```python
from build123d import *

# Parameters (mm, degrees)
BASEHEAD_DEPTH     = 3.5
SKETCH5_R          = 2.5
BASEBODY_DEPTH     = 10
CHAMFER1_SIZE      = 0.25
SCALE1_SCALE       = 0.6
SKETCH1_R          = 1.918221386
CUT_EXTRUDE1_DEPTH = 2


with BuildPart() as part:
    # Sketch2 → BaseHead (new body)
    with BuildSketch(Plane(origin=(0, 0, 0), x_dir=(0, 0, -1), z_dir=(1, 0, 0))):
        Polygon((0, -4.618802154), (4, -2.309401077), (4, 2.309401077), (0, 4.618802154), (-4, 2.309401077), (-4, -2.309401077), align=None)
    extrude(amount=BASEHEAD_DEPTH)

    # Sketch3 → BearingFace (revolve, cut)
    with BuildSketch(Plane.XY, mode=Mode.PRIVATE) as bearingface_sk:
        Polygon((3.5, 4.618802154), (3.5, 3.37), (3, 3.87), (3, 4.618802154), align=None)
    revolve(bearingface_sk.sketch.rotate(Axis((-0.957090588, 0, 0), (1, 0, 0)), 90), axis=Axis((-0.957090588, 0, 0), (1, 0, 0)), mode=Mode.SUBTRACT)

    # Sketch4 → HeadChamfer (revolve, cut)
    with BuildSketch(Plane.XY):
        Polygon((0, 4.618802154), (0.225225565, 4.618802154), (0, 4), align=None)
    revolve(axis=Axis((-0.493528746, 0, 0), (1, 0, 0)), mode=Mode.SUBTRACT)

    # Sketch5 → BaseBody (add)
    with BuildSketch(Plane(origin=(3.5, 0, 0), x_dir=(0, 0, -1), z_dir=(1, 0, 0))):
        with Locations(Location((0, 0, 0), (0, 0, 180))):
            Circle(SKETCH5_R)
    extrude(amount=BASEBODY_DEPTH)

    # Chamfer1
    chamfer1_edges = [part.edges().sort_by_distance(p)[0] for p in [
        (13.5, 0, -2.5),
    ]]
    chamfer(chamfer1_edges, length=CHAMFER1_SIZE)


with BuildPart() as part_1:
    # Scale1: scaled about (5.174356306, 0, 0)
    add(part.part.scale(SCALE1_SCALE).moved(Location((2.069742522, 0, 0))))

    # Sketch1 → Cut-Extrude1 (cut)
    with BuildSketch(Plane(origin=(10.169743001, 0, 0), x_dir=(0, 0, -1), z_dir=(1, 0, 0))):
        Circle(SKETCH1_R)
    extrude(amount=-CUT_EXTRUDE1_DEPTH, mode=Mode.SUBTRACT)


solid = part_1.part
```
CAD build for the part. Positions are in the model's coordinates, mm. Round coordinates to 2 decimals unless told otherwise and drop trailing zeros. Write each loop counter-clockwise with the first axis right and the second up, starting at its lowest first coordinate (ties: lowest second). Pieces come first, ordered by that corner, then holes. Notation, with made-up numbers: (22.25, 30.5) -> (46.25, 30.5) arc R25 ccw to (46.25, 48.5) -> close; hole circle Ø5 at (79, 43.25). An arc over 180 degrees is marked (long way). Answer in a Markdown table with one row per item. Add a question column.
Item 1: Drill centre lines: line 1 (Y direction, x = 6, z = 0.9); line 2 (X direction, y = -1.8, z = -0.1); line 3 (X direction, y = -1.9, z = -1.4). Where is each one in solid material? Low to high. Write a range as from..to.
Item 2: Saw through at B-B, the plane x = 7.25. Write the cut outline in (y, z), then the cut area to 3 significant figures.
Item 3: Mould opens along Z. For faces 1 (the face through (3, 0, -2.4)), 2 (the face through (6.14, -0.45, 1.43)), 3 (the face through (2.96, 2.09, 1.18)) say: pulls with the +Z half, pulls with the -Z half, needs draft (parallel to the pull), parting line crosses it, or undercut.
Item 4: Drop a flat-ended pin along its axis: pin 1 Ø1.5 at (x, y) = (6, 1) entering from +Z. Give the stop position or say it passes through.
Item 5: Saw through at A-A, the plane x = 3.25. Write the cut outline in (y, z).
Findings below:
| question | item | result |
|---|---|---|
| 1 | line 1 | y = -1.2..1.2 |
| 1 | line 2 | x = 2.07..4.17 |
| 1 | line 3 | x = 2.07..3.87 |
| 2 | outline | circle Ø3 at (0, 0) |
| 2 | area | 7.07 mm^2 |
| 3 | face 1 | pulls with the -Z half |
| 3 | face 2 | parting line crosses it |
| 3 | face 3 | pulls with the +Z half |
| 4 | pin 1 | stops at z = 1.48 |
| 5 | outline | (-2.77, 0) -> (-1.39, -2.4) -> (1.39, -2.4) -> (2.77, 0) -> (1.39, 2.4) -> (-1.39, 2.4) -> close |
